from build123d import *

# Parameters (mm, degrees)
BOSS_EXTRUDE1_DEPTH = 1393
SHELL1_T            = -4


with BuildPart() as part:
    # Sketch1 → Boss-Extrude1 (new body)
    with BuildSketch(Plane.XY):
        with BuildLine():
            Line((35, 25), (-35, 25))
            ThreePointArc((-35, 25), (-38.535533906, 23.535533906), (-40, 20))
            Line((-40, 20), (-40, -20))
            ThreePointArc((-40, -20), (-38.535533906, -23.535533906), (-35, -25))
            Line((-35, -25), (35, -25))
            ThreePointArc((35, -25), (38.535533906, -23.535533906), (40, -20))
            Line((40, -20), (40, 20))
            ThreePointArc((40, 20), (38.535533906, 23.535533906), (35, 25))
        make_face()
    extrude(amount=BOSS_EXTRUDE1_DEPTH)

    # Shell1
    shell1_openings = [part.faces().sort_by_distance(p)[0] for p in [
        (0, 0, 1393),
        (0, 0, 0),
    ]]
    offset(amount=SHELL1_T, openings=shell1_openings, kind=Kind.INTERSECTION)


solid = part.part
Could you check a few things on this model? Use its own coordinates, in mm. A direction names the side the tool comes from. Give positions to 0.01 mm unless a question says otherwise; leave off trailing zeros. Write each loop counter-clockwise with the first axis right and the second up, starting at its lowest first coordinate (ties: lowest second). Pieces come first, ordered by that corner, then holes. Notation, with made-up numbers: (4.5, 3.25) -> (60.5, 3.25) arc R21 ccw to (60.5, 21.25) -> close; hole circle Ø11 at (-36, 77). An arc over 180 degrees is marked (long way). Answer as CSV lines item,"result". Start each with the question number.
(1) Please list where these lines run through material, in increasing order: line 1 (Y direction, x = -25, z = 58); line 2 (X direction, y = -6, z = 76.5); line 3 (X direction, y = -20.5, z = 410.5).
(2) I'm going to push flat-ended pins straight in: pin 1 Ø5 at (x, y) = (0, -20) entering from -Z; pin 2 Ø12 at (x, y) = (-28, 5) entering from +Z. Where does each tip first touch, or does it pass through?
(3) If we section it at A-A, the plane y = 12.5: Write out the boundary of the cut face in (x, z), and give its area (3 significant figures).
(4) Which directions (+Z, -Z, +X, -X, +Y, -Y) give clear straight access to the entire face, cutting with the end or side of a thin tool? Please do faces 4 (the face through (-3, -22, 1393)), 5 (the face through (0, 21, 687)).
(5) If we section it at B-B, the plane z = 623: Write out the boundary of the cut face in (x, y), and give its area (3 significant figures).
(6) If we mould it in two halves opening along X, with no side actions, what happens to faces 1 (the face through (-36, 0, 687)), 2 (the face through (-40, 0, 687)), 3 (the face through (0, 25, 687))? For each: +X half, -X half, draft (parallel to the pull), parting line (faces both ways), or undercut.
(7) If we section it at C-C, the plane x = 20.5: Write out the boundary of the cut face in (y, z), and give its area (3 significant figures).
Answer list:
1,line 1,"-25 to -21, 21 to 25"
1,line 2,"-40 to -36, 36 to 40"
1,line 3,"-39.97 to -35.87, 35.87 to 39.97"
2,pin 1,"z = 0"
2,pin 2,"through"
3,outline,"(-40, 0) -> (-36, 0) -> (-36, 1393) -> (-40, 1393) -> close; (36, 0) -> (40, 0) -> (40, 1393) -> (36, 1393) -> close"
3,area,"11,100 mm^2"
4,face 4,"+Z, +X, -X, +Y, -Y"
4,face 5,"+Z, -Z"
5,outline,"(-40, -20) arc R5 ccw to (-35, -25) -> (35, -25) arc R5 ccw to (40, -20) -> (40, 20) arc R5 ccw to (35, 25) -> (-35, 25) arc R5 ccw to (-40, 20) -> close; hole (-36, -20) arc R1 ccw to (-35, -21) -> (35, -21) arc R1 ccw to (36, -20) -> (36, 20) arc R1 ccw to (35, 21) -> (-35, 21) arc R1 ccw to (-36, 20) -> close"
5,area,"955 mm^2"
6,face 1,"undercut"
6,face 2,"-X half"
6,face 3,"draft"
7,outline,"(-25, 0) -> (-21, 0) -> (-21, 1393) -> (-25, 1393) -> close; (21, 0) -> (25, 0) -> (25, 1393) -> (21, 1393) -> close"
7,area,"11,100 mm^2"
